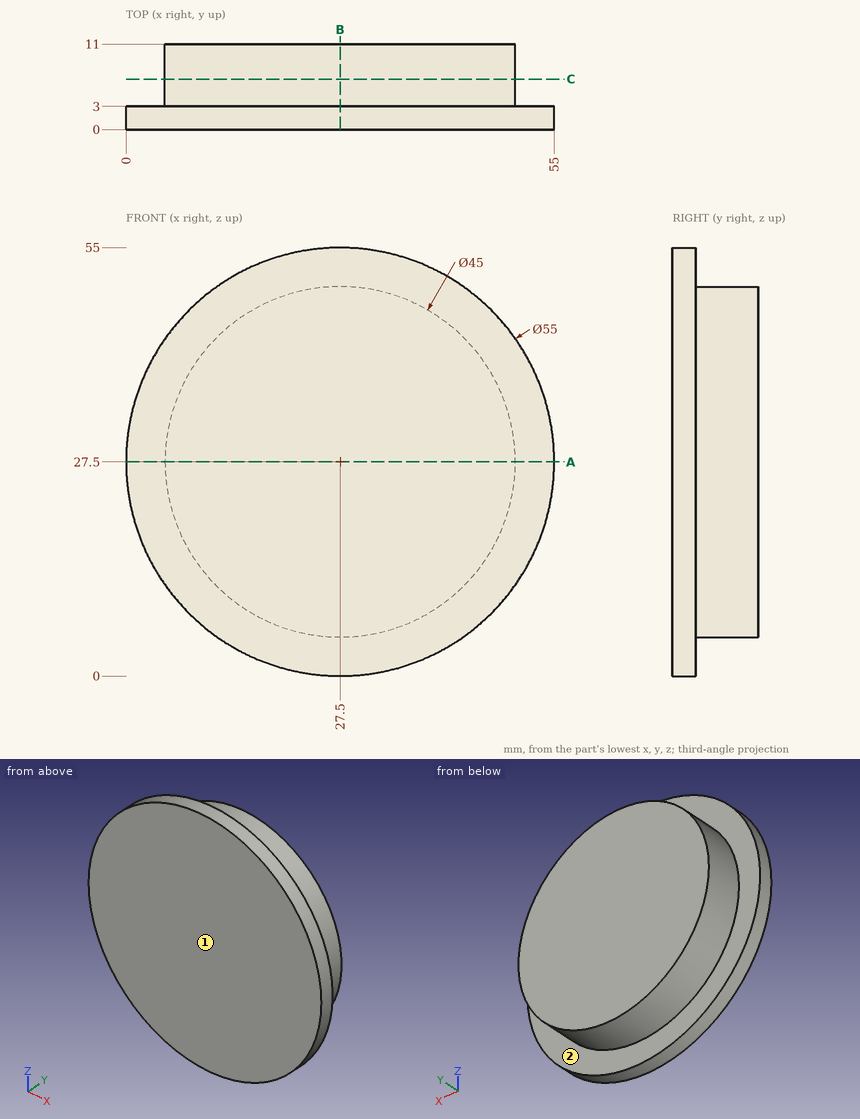
For this review, use the dimensioned drawing (mm, ordinates from the lowest corner) and the shaded views. A direction names the side the tool comes from. Round coordinates to 2 decimals unless told otherwise and drop trailing zeros. Write each loop counter-clockwise with the first axis right and the second up, starting at its lowest first coordinate (ties: lowest second). Pieces come first, ordered by that corner, then holes. Notation, with made-up numbers: (-9, -17) - (23, -17) arc R19 ccw to (23, 6) - close; hole circle Ø9 at (15.25, 85). An arc over 180 degrees is marked (long way). One line per item, written item: value. Start each with the question number.
1. Consider section C-C on y = 6.5. Write out the cut boundary in (x, z).
2. Clearance check with flat-ended pins moving along their axes: P1, Ø1, axis at y = 9, z = 45.5, coming from the -X side; P2, Ø5, axis at x = 12, y = 2, coming from the +Z side; P3, Ø3, axis at x = 47.5, z = 8, coming from the +Y side. State where each tip first meets the part, or that it passes through.
3. Consider section A-A on z = 27.5. Write out the cut boundary in (x, y), and give its area (3 significant figures).
4. To check wall thickness, follow L1, parallel to Y at x = 3, z = 38; L2, parallel to X at y = 9, z = 34.5; L3, parallel to Z at x = 47.5, y = 7.25. State the ranges of each line that lie inside material, in increasing order. Write a range as from..to.
5. Consider section B-B on x = 27.5. Write out the cut boundary in (y, z), and give its area (3 significant figures).
6. Machinability: for the marked faces 1 and 2, which of the approach directions +Z, -Z, +X, -X, +Y, -Y give a long, thin tool a straight path to every point of the face, cutting with its end or side? Answer none if there is none.
Checks:
1. outline: circle Ø45 at (27.5, 27.5)
2. P1: stops at x = 13.36
2. P2: stops at z = 51.73
2. P3: stops at y = 3
3. outline: (0, 0) - (55, 0) - (55, 3) - (50, 3) - (50, 11) - (5, 11) - (5, 3) - (0, 3) - close
3. area: 525 mm^2
4. L1: y = 0..3
4. L2: x = 6.12..48.88
4. L3: z = 17.19..37.81
5. outline: (0, 0) - (3, 0) - (3, 5) - (11, 5) - (11, 50) - (3, 50) - (3, 55) - (0, 55) - close
5. area: 525 mm^2
6. face 1: +Z, -Z, +X, -X, -Y
6. face 2: +Y
